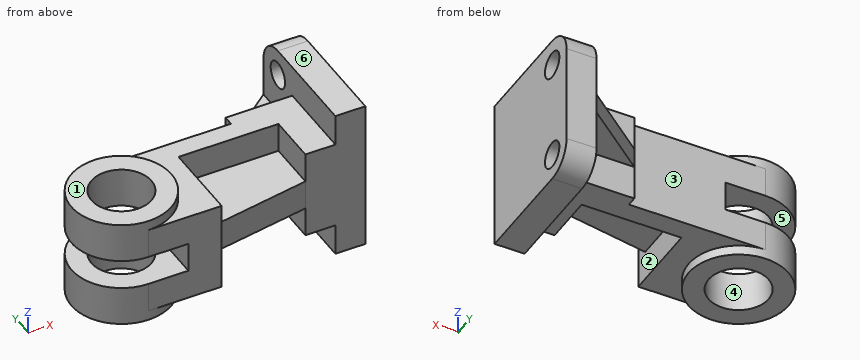
from build123d import *

# Parameters (mm, degrees)
HUB_PROFILE_SKETCH_R         = 30
HUB_60_DEPTH                 = 24
HUB_EXTENSION_SKETCH_R       = 30
HUB_EXTENSION_60_DEPTH       = 24
HUB_BORE_SKETCH_R            = 18
HUB_BORE_36_DEPTH            = 98
ARM_START                    = -54
ARM_BODY_DEPTH               = 54
CLEVIS_SLOT_SKETCH_W         = 24
CLEVIS_SLOT_SKETCH_H         = 18
CLEVIS_SLOT_24MM_DEPTH       = 96
SLOT_PAD_SKETCH_W            = 18
SLOT_PAD_SKETCH_H            = 60
SLOT_PAD_5MM_DEPTH           = 5
RIB_BASE_PAD_SKETCH_W        = 40
RIB_BASE_PAD_SKETCH_H        = 54
RIB_BASE_PAD_DEPTH           = 6
MOUNTING_FLANGE_SKETCH_W     = 18
MOUNTING_FLANGE_SKETCH_H     = 80
MOUNTING_FLANGE_DEPTH        = 46
FLANGE_CORNER_FILLET_R16_A_R = 16
FLANGE_CORNER_FILLET_R16_B_R = 16
FLANGE_HOLES_SKETCH_R        = 8
FLANGE_HOLES_2X_16_DEPTH     = 92
FLANGE_RIB_12MM_REACH        = 164.296
FLANGE_RIB_SKETCH_WALL_W     = 377.817045558
FLANGE_RIB_SKETCH_WALL_H     = 12
ARM_RELIEF_CUT_DEPTH         = 92
ARM_RIB_18MM_REACH           = 164.296
ARM_RIB_SKETCH_WALL_W        = 432.138250074
ARM_RIB_SKETCH_WALL_H        = 18


with BuildPart() as part:
    # Hub Profile Sketch → Hub Ø60 (new body)
    with BuildSketch(Plane.XY):
        Circle(HUB_PROFILE_SKETCH_R)
    extrude(amount=HUB_60_DEPTH)


with BuildPart() as body_2:
    # Hub Extension Sketch → Hub Extension Ø60 (new body)
    with BuildSketch(Plane(origin=(0, 0, -18), x_dir=(-1, 0, 0), z_dir=(0, 0, -1))):
        with Locations(Location((0, 0, 0), (0, 0, 180))):
            Circle(HUB_EXTENSION_SKETCH_R)
    extrude(amount=HUB_EXTENSION_60_DEPTH)


with BuildPart() as hub_bore_36_tool:
    # Hub Bore Sketch → Hub Bore Ø36 (new body)
    with BuildSketch(Plane.XY.offset(24)):
        Circle(HUB_BORE_SKETCH_R)
    extrude(amount=-HUB_BORE_36_DEPTH)


with BuildPart() as part_1:
    add(part.part)

    # Hub Bore Ø36: cut by hub_bore_36_tool
    add(hub_bore_36_tool.part, mode=Mode.SUBTRACT)



with BuildPart() as body_2_1:
    add(body_2.part)

    # Hub Bore Ø36: cut by hub_bore_36_tool
    add(hub_bore_36_tool.part, mode=Mode.SUBTRACT)


with BuildPart() as part_2:
    add(part_1.part)

    add(body_2_1.part)  # Arm Body merges body 2
    # Arm Profile Sketch → Arm Body (add)
    with BuildSketch(Plane.XY.offset(18).offset(ARM_START)):
        with BuildLine():
            Line((0, 30), (122, 30))
            Line((122, 30), (122, -30))
            Line((122, -30), (0, -30))
            ThreePointArc((0, -30), (30, 0), (0, 30))
        make_face()
    extrude(amount=ARM_BODY_DEPTH)

    # Clevis Slot Sketch → Clevis Slot 24mm (cut)
    with BuildSketch(Plane(origin=(0, 30, 0), x_dir=(1, 0, 0), z_dir=(0, 1, 0))):
        with Locations((12, 9)):
            Rectangle(CLEVIS_SLOT_SKETCH_W, CLEVIS_SLOT_SKETCH_H)
    extrude(amount=-CLEVIS_SLOT_24MM_DEPTH, mode=Mode.SUBTRACT)

    # Slot Pad Sketch → Slot Pad 5mm (add)
    with BuildSketch(Plane.ZY.offset(-24)):
        with Locations((-9, 0)):
            Rectangle(SLOT_PAD_SKETCH_W, SLOT_PAD_SKETCH_H)
    extrude(amount=-SLOT_PAD_5MM_DEPTH)

    # Rib Base Pad Sketch → Rib Base Pad (add)
    with BuildSketch(Plane(origin=(0, 30, 0), x_dir=(1, 0, 0), z_dir=(0, 1, 0))):
        with Locations((102, 9)):
            Rectangle(RIB_BASE_PAD_SKETCH_W, RIB_BASE_PAD_SKETCH_H)
    extrude(amount=RIB_BASE_PAD_DEPTH)

    # Mounting Flange Sketch → Mounting Flange (add, symmetric)
    with BuildSketch(Plane(origin=(0, 0, -9), x_dir=(-1, 0, 0), z_dir=(0, 0, -1))):
        with Locations((-131, 28)):
            Rectangle(MOUNTING_FLANGE_SKETCH_W, MOUNTING_FLANGE_SKETCH_H)
    extrude(amount=MOUNTING_FLANGE_DEPTH, both=True)

    # Flange Corner Fillet R16 A
    flange_corner_fillet_r16_a_edges = [part_2.edges().sort_by_distance(p)[0] for p in [
        (131, 68, 37),
    ]]
    fillet(flange_corner_fillet_r16_a_edges, radius=FLANGE_CORNER_FILLET_R16_A_R)

    # Flange Corner Fillet R16 B
    flange_corner_fillet_r16_b_edges = [part_2.edges().sort_by_distance(p)[0] for p in [
        (131, 68, -55),
    ]]
    fillet(flange_corner_fillet_r16_b_edges, radius=FLANGE_CORNER_FILLET_R16_B_R)

    # Flange Holes Sketch → Flange Holes 2xØ16 (cut)
    with BuildSketch(Plane.ZY.offset(-122)):
        with Locations((21, 52)):
            Circle(FLANGE_HOLES_SKETCH_R)
        with Locations((-39, 52)):
            Circle(FLANGE_HOLES_SKETCH_R)
    extrude(amount=-FLANGE_HOLES_2X_16_DEPTH, mode=Mode.SUBTRACT)

    # Flange Rib Sketch wall → Flange Rib 12mm (add, up to next)
    with BuildSketch(Plane(origin=(102, 52, -9), x_dir=(0.780868809443, 0.624695047554, 0), z_dir=(0.624695047554, -0.780868809443, 0)), mode=Mode.PRIVATE) as flange_rib_12mm_sk1:
        Rectangle(FLANGE_RIB_SKETCH_WALL_W, FLANGE_RIB_SKETCH_WALL_H)
    flange_rib_12mm_tool1 = extrude(flange_rib_12mm_sk1.sketch, amount=FLANGE_RIB_12MM_REACH, mode=Mode.PRIVATE) - part_2.part
    add(flange_rib_12mm_tool1.solids().sort_by_distance((102, 52, -9))[0])

    # Arm Relief Sketch → Arm Relief Cut (cut)
    with BuildSketch(Plane.XY.offset(18)):
        Polygon((104, 18), (104, -12), (44, -30), (44, 18), align=None)
        Polygon((122, -30), (122, -12), (104, -12), (44, -30), align=None)
    extrude(amount=-ARM_RELIEF_CUT_DEPTH, mode=Mode.SUBTRACT)

    # Arm Rib Sketch wall → Arm Rib 18mm (add, up to next)
    with BuildSketch(Plane(origin=(52, -21, -9), x_dir=(0.985350505855, 0.170541433706, 0), z_dir=(0.170541433706, -0.985350505855, 0)), mode=Mode.PRIVATE) as arm_rib_18mm_sk1:
        Rectangle(ARM_RIB_SKETCH_WALL_W, ARM_RIB_SKETCH_WALL_H)
    arm_rib_18mm_tool1 = extrude(arm_rib_18mm_sk1.sketch, amount=-ARM_RIB_18MM_REACH, mode=Mode.PRIVATE) - part_2.part
    add(arm_rib_18mm_tool1.solids().sort_by_distance((52, -21, -9))[0])


solid = part_2.part
Can you work these out from the model? Positions are in its coordinate system, mm. Face numbers are marked on the shaded views. A direction names the side the tool comes from. Give positions to 0.01 mm unless a question says otherwise; leave off trailing zeros. Write each loop counter-clockwise with the first axis right and the second up, starting at its lowest first coordinate (ties: lowest second). Pieces come first, ordered by that corner, then holes. Notation, with made-up numbers: M 68.25,41.5 L 102.25,41.5 A9 ccw 102.25,49.5 Z; hole C 5.25,-39.75 d11. An arc over 180 degrees is marked long. Answer in a Markdown table with one row per item. Add a question column.
Item 1: Imagine slicing it at B-B, the plane x = -10.5. Write out the boundary of the cut face in (y, z).
Item 2: We'd pull the mould along Z, two halves only. Please class the marked faces 4, 5 and 6: released by +Z, released by -Z, zero draft, split by the parting line, or undercut.
Item 3: Imagine slicing it at D-D, the plane y = 47. Write out the boundary of the cut face in (x, z) (3 decimals).
Item 4: Imagine slicing it at C-C, the plane z = -26. Write out the boundary of the cut face in (x, y), plus the area to 3 significant figures.
Item 5: On a 3-axis mill with a long thin cutter (end or side, diameter ignored), from which of +Z, -Z, +X, -X, +Y, -Y can I reach the whole of each face in a straight line? I mean the marked faces 1, 2 and 3. Say none if no direction works.
Item 6: For pin 1 Ø6 at (x, z) = (90, -35.5) entering from +Y; pin 2 Ø9 at (y, z) = (1, -23) entering from -X; pin 3 Ø0.5 at (x, y) = (29.5, -0.5) entering from +Z; pin 4 Ø12 at (x, z) = (100.5, 26) entering from -Y, each with a flat end and sliding along its axis, tell me the tip position at first contact or that it passes through.
Item 7: Please list where these lines run through material, in increasing order: L1, parallel to X at y = 0, z = -23; L2, parallel to Z at x = 3.5, y = 25; L3, parallel to X at y = -10.5, z = 17.
Item 8: Imagine slicing it at A-A, the plane y = 0. State how many separate pieces and enclosed holes the cut face has, plus the area to 3 significant figures.
Evaluation:
| question | item | result |
|---|---|---|
| 1 | outline | M -28.1,-42 L -14.62,-42 L -14.62,-18 L -28.1,-18 Z; M -28.1,0 L -14.62,0 L -14.62,24 L -28.1,24 Z; M 14.62,-42 L 28.1,-42 L 28.1,-18 L 14.62,-18 Z; M 14.62,0 L 28.1,0 L 28.1,24 L 14.62,24 Z |
| 2 | face 4 | zero draft |
| 2 | face 5 | undercut |
| 2 | face 6 | released by +Z |
| 3 | outline | M 95.75,-15 L 122,-15 L 122,-32.755 L 140,-32.755 L 140,14.755 L 122,14.755 L 122,-3 L 95.75,-3 Z; M 122,-55 L 140,-55 L 140,-45.245 L 122,-45.245 Z; M 122,27.245 L 140,27.245 L 140,37 L 122,37 Z |
| 4 | outline | M 0,-30 L 44,-30 L 44,18 L 104,18 L 104,-12 L 140,-12 L 140,68 L 122,68 L 122,36 L 82,36 L 82,30 L 0,30 A30 ccw Z; hole C 0,0 d36 |
| 4 | area | 6,190 mm² |
| 5 | face 1 | +Z, -X, +Y, -Y |
| 5 | face 2 | -Y |
| 5 | face 3 | +Z, -Z, -X, +Y |
| 6 | pin 1 | stops at y = 36 |
| 6 | pin 2 | stops at x = -30 |
| 6 | pin 3 | stops at z = 24 |
| 6 | pin 4 | passes through |
| 7 | L1 | x = -30 to -18, 18 to 44, 104 to 140 |
| 7 | L2 | z = -42 to -18, 0 to 24 |
| 7 | L3 | x = -28.1 to -14.62, 14.62 to 44, 104 to 140 |
| 8 | separate pieces | 3 |
| 8 | enclosed holes | 1 |
| 8 | area | 5,710 mm² |
